```python
from build123d import *

# Parameters (mm, degrees)
SKETCH1_R           = 10
BOSS_EXTRUDE1_DEPTH = 30
SKETCH2_R           = 12.5
BOSS_EXTRUDE2_DEPTH = 20
SKETCH3_R           = 5
BOSS_EXTRUDE3_DEPTH = 20


with BuildPart() as part:
    # Sketch1 → Boss-Extrude1 (new body)
    with BuildSketch(Plane.XY):
        Circle(SKETCH1_R)
    extrude(amount=BOSS_EXTRUDE1_DEPTH)

    # Sketch2 → Boss-Extrude2 (add)
    with BuildSketch(Plane.XY.offset(30)):
        Circle(SKETCH2_R)
    extrude(amount=BOSS_EXTRUDE2_DEPTH)

    # Sketch3 → Boss-Extrude3 (add)
    with BuildSketch(Plane.XY.offset(50)):
        Circle(SKETCH3_R)
    extrude(amount=BOSS_EXTRUDE3_DEPTH)


solid = part.part
```
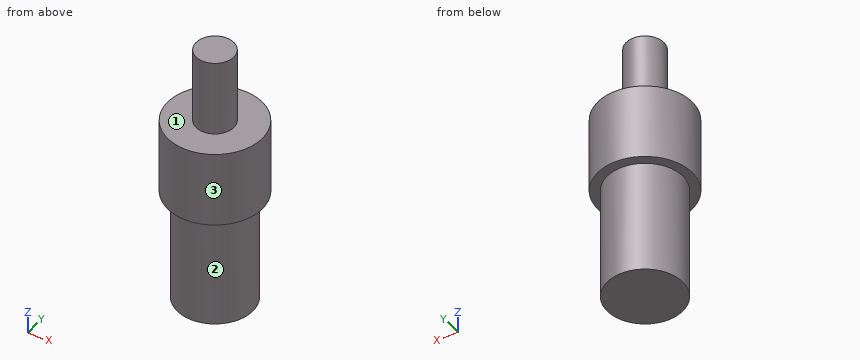
The model under review builds one solid part; all positions refer to its coordinate system, in mm. Face numbers are marked on the shaded views. A direction names the side the tool comes from. Round coordinates to 2 decimals unless told otherwise and drop trailing zeros. Loops run counter-clockwise (first coordinate to the right, second up) from the corner with the lowest first, then second, coordinate; pieces in that order, holes last. Notation, with made-up numbers: M 41,-20 L 79,-20 A3 ccw 79,-15 Z; hole C 88,-37.75 d4. An arc over 180 degrees is marked long. Put each result on its own line as item: value.
Q1. Consider section A-A, the plane y = 0. Give the boundary of the cut face in (x, z).
Result set:
outline: M -12.5,30 L -10,30 L -10,0 L 10,0 L 10,30 L 12.5,30 L 12.5,50 L 5,50 L 5,70 L -5,70 L -5,50 L -12.5,50 Z
Q2. Consider section D-D, the plane y = -6. Give the boundary of the cut face in (x, z), then the cut area to 3 significant figures.
Result set:
outline: M -10.97,30 L -8,30 L -8,0 L 8,0 L 8,30 L 10.97,30 L 10.97,50 L -10.97,50 Z
area: 919 mm²
Q3. Consider section C-C, the plane z = 33.5. Give the boundary of the cut face in (x, y), then the cut area to 3 significant figures.
Result set:
outline: C 0,0 d25
area: 491 mm²
Q4. To check wall thickness, follow L1, parallel to Z at x = -7.75, y = 8; L2, parallel to Y at x = 0.5, z = 19; L3, parallel to Z at x = 8.25, y = 5.25. State the ranges of each line that lie inside material, in increasing order.
Result set:
L1: z = 30 to 50
L2: y = -9.99 to 9.99
L3: z = 0 to 50
Q5. For pin 1 (1 mm diameter, centred on x = 2.5, z = 44, fed in from -Y); pin 2 (4 mm diameter, centred on y = -5.5, z = 56.5, fed in from +X); pin 3 (6 mm diameter, centred on y = 3, z = 8, fed in from +X), all flat-tipped, find the tip position at first contact; note any pin that passes through.
Result set:
pin 1: stops at y = -12.34
pin 2: stops at x = 3.57
pin 3: stops at x = 10
Q6. Machinability: for the marked faces 1, 2 and 3, which of the approach directions +Z, -Z, +X, -X, +Y, -Y give a long, thin tool a straight path to every point of the face, cutting with its end or side? Answer none if there is none.
Result set:
face 1: +Z
face 2: -Z
face 3: +Z, -Z
